CAD build for the part. Positions are in the model's coordinates, mm. A direction names the side the tool comes from. Round coordinates to 2 decimals unless told otherwise and drop trailing zeros. Write each loop counter-clockwise with the first axis right and the second up, starting at its lowest first coordinate (ties: lowest second). Pieces come first, ordered by that corner, then holes. Notation, with made-up numbers: (76.25, -4.5) - (86.25, -4.5) arc R8 cw to (86.25, 6.5) - close; hole circle Ø8 at (22, 21.5). An arc over 180 degrees is marked (long way). Put each result on its own line as item: value. Start each with the question number.
Item 1: Mould opens along X. For faces 1 (the flat face through (50, 25, 190)), 2 (the flat face through (25, 47, 190)), 3 (the flat face through (2.7, 25.1, 400)) say: released by +X, released by -X, zero draft, split by the parting line, or undercut.
Item 2: Cut at A-A (x = 36.5). Give the cut face in (y, z).
Item 3: Drill centre line: line 1 (X direction, y = 42, z = 147). Where is it in solid material? Low to high. Write a range as from..to.
Item 4: 3-axis set-ups, long thin cutter, end or side, ignore diameter. For faces 4 (the flat face through (0, 25, 190)), 5 (the flat face through (25, 3, 190)): which of +Z, -Z, +X, -X, +Y, -Y reach the whole face in a straight line?
Item 5: Cut at C-C (z = 9). Give the cut face in (x, y), and give its area (3 significant figures).
```python
from build123d import *

# Parameters (mm, degrees)
SKETCH_1_W          = 50
SKETCH_1_H          = 50
SKETCH_1_W_2        = 44
SKETCH_1_H_2        = 44
EXTRUDE_1_DEPTH     = 400
SKETCH_2_W          = 50
SKETCH_2_H          = 50
SKETCH_2_W_2        = 44
SKETCH_2_H_2        = 44
CUT_EXTRUDE_1_DEPTH = 25
SKETCH_3_W          = 50
SKETCH_3_H          = 50
SKETCH_3_W_2        = 44
SKETCH_3_H_2        = 44
EXTRUDE_2_DEPTH     = 50


with BuildPart() as part:
    # 草图1 → 凸台-拉伸1 (new body)
    with BuildSketch(Plane.XY):
        with Locations((25, 25)):
            Rectangle(SKETCH_1_W, SKETCH_1_H)
        with Locations((25, 25)):
            Rectangle(SKETCH_1_W_2, SKETCH_1_H_2, mode=Mode.SUBTRACT)
    extrude(amount=EXTRUDE_1_DEPTH)

    # 草图2 → 切除-拉伸1 (cut)
    with BuildSketch(Plane(origin=(0, 0, 0), x_dir=(-1, 0, 0), z_dir=(0, 0, -1))):
        with Locations((-25, 25)):
            Rectangle(SKETCH_2_W, SKETCH_2_H)
        with Locations((-25, 25)):
            Rectangle(SKETCH_2_W_2, SKETCH_2_H_2, mode=Mode.SUBTRACT)
    extrude(amount=-CUT_EXTRUDE_1_DEPTH, mode=Mode.SUBTRACT)

    # 草图3 → 凸台-拉伸2 (add)
    with BuildSketch(Plane(origin=(0, 0, 25), x_dir=(-1, 0, 0), z_dir=(0, 0, -1))):
        with Locations((-25, 25)):
            Rectangle(SKETCH_3_W, SKETCH_3_H)
        with Locations((-25, 25)):
            Rectangle(SKETCH_3_W_2, SKETCH_3_H_2, mode=Mode.SUBTRACT)
    extrude(amount=EXTRUDE_2_DEPTH)


solid = part.part
```
Output values:
1. face 1: released by +X
1. face 2: undercut
1. face 3: zero draft
2. outline: (0, -25) - (3, -25) - (3, 400) - (0, 400) - close; (47, -25) - (50, -25) - (50, 400) - (47, 400) - close
3. line 1: 0..3, 47..50
4. face 4: +Z, -Z, -X, +Y, -Y
4. face 5: +Z, -Z
5. outline: (0, 0) - (50, 0) - (50, 50) - (0, 50) - close; hole (3, 3) - (47, 3) - (47, 47) - (3, 47) - close
5. area: 564 mm2
